Part model, mm, in its own coordinate system. A direction names the side the tool comes from. Coordinates: 2 decimals unless noted, no trailing zeros. Write each loop counter-clockwise with the first axis right and the second up, starting at its lowest first coordinate (ties: lowest second). Pieces come first, ordered by that corner, then holes. Notation, with made-up numbers: (-26.75, -17) -> (21.25, -17) arc R19 ccw to (21.25, 6) -> close; hole circle Ø10 at (-39.5, 18). An arc over 180 degrees is marked (long way). Write item = value, one per line. Start each with the question number.
Q1. Band-saw the part on A-A, the plane y = 41.5. List the corners of the cut face in (x, z).
Q2. Probe line 1 (X direction, y = 0, z = 8); line 2 (X direction, y = 54, z = 27.5); line 3 (Y direction, x = 11, z = 19). List the from-to ranges inside material, lowest first.
Q3. Band-saw the part on B-B, the plane z = 19. List the corners of the cut face in (x, y), plus the area to 4 significant figures.
Q4. Tool access for faces 1 (the flat face through (-11, 21, 38)), 2 (the flat face through (-7, 51, 19)), 3 (the flat face through (105, -53, 18)): list every direction of +Z, -Z, +X, -X, +Y, -Y with a clear straight run to the whole face (end or side of a thin tool).
Q5. Band-saw the part on D-D, the plane z = -8.5. List the corners of the cut face in (x, y), plus the area to 3 significant figures.
Q6. Band-saw the part on C-C, the plane z = 36. List the corners of the cut face in (x, y).
Q7. Pin check, flat tips, straight feed: P1, Ø17, axis at y = -61.5, z = 32.5, coming from the +X side; P2, Ø1, axis at y = -1, z = 37, coming from the -X side; P3, Ø8, axis at y = -42, z = -1, coming from the -X side. Stop position of each tip, or through.
Q8. Pull direction Y, two halves, no side cores. Call faces 4 (the cylindrical face through (10.94, 66.94, 19.91)), 5 (the cylindrical face through (-0.91, -22.98, 18.73)), 6 (the flat face through (98, -70.036, 18)), 7 (the flat face through (7, 51, 19)): released by +Y, released by -Y, zero draft, split by the parting line, or undercut.
from build123d import *

# Parameters (mm, degrees)
CLAMP_RING_SKETCH_46_62_R   = 31
CLAMP_RING_SKETCH_46_62_R_2 = 23
CLAMP_RING_62X38_DEPTH      = 38
RING_CUT_DEPTH              = 38
CLEVIS_LUG_SKETCH_R         = 7
CLEVIS_LUG_DEPTH            = 8
ANGLE_BRACKET_DEPTH         = 32.5
SUPPORT_WEB_DEPTH           = 5


with BuildPart() as part:
    # Clamp Ring Sketch Ø46-Ø62 → Clamp Ring Ø62x38 (new body)
    with BuildSketch(Plane.XY):
        Circle(CLAMP_RING_SKETCH_46_62_R)
        Circle(CLAMP_RING_SKETCH_46_62_R_2, mode=Mode.SUBTRACT)
    extrude(amount=CLAMP_RING_62X38_DEPTH)

    # Ring Cut Sketch → Ring Cut (cut)
    with BuildSketch(Plane.XY.offset(38)):
        Polygon((0, 0), (-7, 0), (-7, 40.569348476), (7, 40.569348476), (7, 0), align=None)
    extrude(amount=-RING_CUT_DEPTH, mode=Mode.SUBTRACT)

    # Clevis Lug Sketch → Clevis Lug (add)
    with BuildSketch(Plane(origin=(7, 0, 0), x_dir=(0, 0, -1), z_dir=(1, 0, 0))):
        with BuildLine():
            Line((-38, 60), (-38, 21.9089023))
            Line((-38, 21.9089023), (0, 21.9089023))
            Line((0, 21.9089023), (0, 60))
            ThreePointArc((0, 60), (-19, 79), (-38, 60))
        make_face()
        with Locations((-19, 60)):
            Circle(CLEVIS_LUG_SKETCH_R, mode=Mode.SUBTRACT)
    clevis_lug = extrude(amount=CLEVIS_LUG_DEPTH)

    # Clevis Lug Mirror: Clevis Lug across plane
    add(clevis_lug.mirror(Plane(origin=(0, 0, 0), x_dir=(0, 0, 1), z_dir=(1, 0, 0))))



with BuildPart() as body_2:
    # Angle Bracket Sketch → Angle Bracket (new, symmetric)
    with BuildSketch(Plane.XY.offset(18)):
        Polygon((90, -70.036000309), (105, -70.036000309), (105, -36.009933812), (142, -36.009933812), (142, -21.009933812), (90, -21.009933812), align=None)
    extrude(amount=ANGLE_BRACKET_DEPTH, both=True)


with BuildPart() as part_1:
    add(part.part)

    add(body_2.part)  # Support Web merges body 2
    # Support Web Sketch 60deg → Support Web (add, symmetric)
    with BuildSketch(Plane.XY.offset(18)):
        with BuildLine():
            Line((90, -70.036000309), (0, -31))
            ThreePointArc((0, -31), (26.825849969, -15.536208463), (26.888515957, 15.427498489))
            Line((26.888515957, 15.427498489), (90, -21.009933812))
            Line((90, -21.009933812), (142, -21.009933812))
            Line((142, -21.009933812), (142, -36.009933812))
            Line((142, -36.009933812), (105, -36.009933812))
            Line((105, -36.009933812), (105, -70.036000309))
            Line((105, -70.036000309), (90, -70.036000309))
        make_face()
    extrude(amount=SUPPORT_WEB_DEPTH, both=True)


solid = part_1.part
Ans:
q1.outline = (-15, 0) -> (-7, 0) -> (-7, 38) -> (-15, 38) -> close; (7, 0) -> (15, 0) -> (15, 38) -> (7, 38) -> close
q2.line_1 = -31 to -23, 23 to 31
q2.line_2 = -15 to -7, 7 to 15
q2.line_3 = -35.77 to -20.2, 20.2 to 53, 67 to 79
q3.outline = (-15, 27.13) arc R31 ccw to (0, -31) -> (90, -70.04) -> (105, -70.04) -> (105, -36.01) -> (142, -36.01) -> (142, -21.01) -> (90, -21.01) -> (26.89, 15.43) arc R31 ccw to (15, 27.13) -> (15, 53) -> (7, 53) -> (7, 21.91) arc R23 cw (long way) to (-7, 21.91) -> (-7, 53) -> (-15, 53) -> close; (-15, 67) -> (-7, 67) -> (-7, 79) -> (-15, 79) -> close; (7, 67) -> (15, 67) -> (15, 79) -> (7, 79) -> close
q3.area = 6,685 mm2
q4.face_1 = +Z, -X, +Y, -Y
q4.face_2 = +Z, -Z, +Y
q4.face_3 = +Z, -Z, +X, -Y
q5.outline = (90, -70.04) -> (105, -70.04) -> (105, -36.01) -> (142, -36.01) -> (142, -21.01) -> (90, -21.01) -> close
q5.area = 1,290 mm2
q6.outline = (-15, 27.13) arc R31 ccw (long way) to (15, 27.13) -> (15, 68.49) -> (7, 68.49) -> (7, 21.91) arc R23 cw (long way) to (-7, 21.91) -> (-7, 68.49) -> (-15, 68.49) -> close; (90, -70.04) -> (105, -70.04) -> (105, -36.01) -> (142, -36.01) -> (142, -21.01) -> (90, -21.01) -> close
q7.P1 = 105
q7.P2 = -31
q7.P3 = 90
q8.face_4 = undercut
q8.face_5 = undercut
q8.face_6 = released by -Y
q8.face_7 = zero draft
